For this review, use the dimensioned drawing (mm, ordinates from the lowest corner) and the shaded views. A direction names the side the tool comes from. Coordinates: 2 decimals unless noted, no trailing zeros. Write each loop counter-clockwise with the first axis right and the second up, starting at its lowest first coordinate (ties: lowest second). Pieces come first, ordered by that corner, then holes. Notation, with made-up numbers: M -12.75,36.5 L -5.75,36.5 A19 ccw -5.75,69.5 Z; hole C -15.75,-33.75 d5. An arc over 180 degrees is marked long. One line per question, with ' | ' between items.
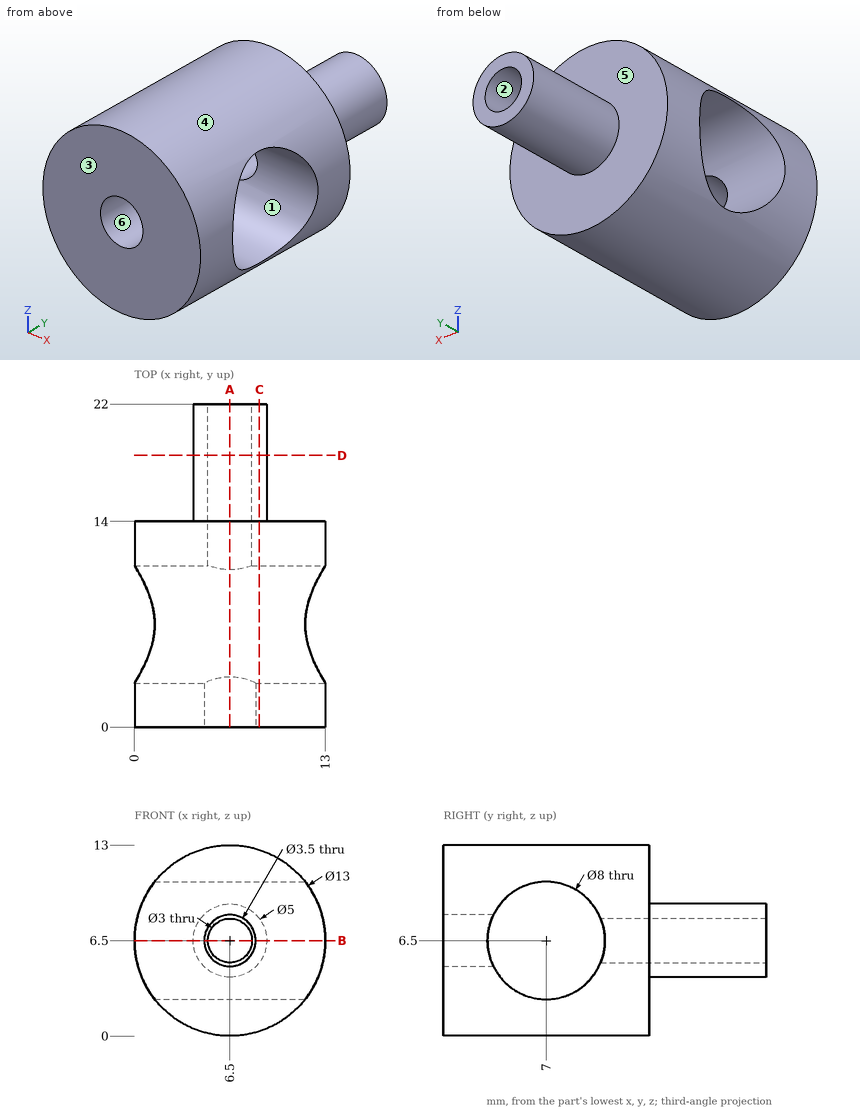
1. Draft analysis for pull direction Y (two halves, no side actions). For the marked faces 1, 2 and 3, state which applies: pulls with the +Y half, pulls with the -Y half, needs draft (parallel to the pull), parting line crosses it, or undercut.
Answer sheet:
face 1: undercut | face 2: needs draft | face 3: pulls with the -Y half
2. Insertion check: pin 1 Ø1 at (x, z) = (11.5, 3) entering from +Y; pin 2 Ø5 at (y, z) = (7, 6.5) entering from -X; pin 3 Ø1.5 at (x, y) = (7.5, 11.5) entering from -Z. Each pin has a flat end and moves straight along its axis. Give the tip position at first contact, or say it passes through.
Answer sheet:
pin 1: y = 14 | pin 2: through | pin 3: z = 0
3. Take a section at C-C (x = 8.5). Write out the cut boundary in (y, z).
Answer sheet:
outline: M 0,0.32 L 14,0.32 L 14,5 L 22,5 L 22,8 L 14,8 L 14,12.68 L 0,12.68 Z; hole C 7,6.5 d8
4. To check wall thickness, follow line 1 along Y through (x, z) = (3.5, 6.5); line 2 along X through (y, z) = (1.15, 6.5); line 3 along Y through (x, z) = (2.5, 3.5). State the ranges of each line that lie inside material, in increasing order. Write a range as [from, to].
Answer sheet:
line 1: [0, 3], [11, 14] | line 2: [0, 4.75], [8.25, 13] | line 3: [0, 4.35], [9.65, 14]
5. Take a section at D-D (y = 18.5). Write out the cut boundary in (x, z), then the cut area to 3 significant figures.
Answer sheet:
outline: C 6.5,6.5 d5; hole C 6.5,6.5 d3 | area: 12.6 mm^2
6. Tool access review of the marked faces 4, 5 and 6: name each direction out of +Z, -Z, +X, -X, +Y, -Y from which nothing blocks a thin tool from reaching the whole face with its end or side.
Answer sheet:
face 4: +Y, -Y | face 5: +Y | face 6: -Y
7. Take a section at A-A (x = 6.5). Write out the cut boundary in (y, z).
Answer sheet:
outline: M 0,0 L 14,0 L 14,4 L 22,4 L 22,5 L 10.71,5 A4 cw 3.4,4.75 L 0,4.75 Z; M 0,8.25 L 3.4,8.25 A4 cw 10.71,8 L 22,8 L 22,9 L 14,9 L 14,13 L 0,13 Z
8. Take a section at B-B (z = 6.5). Write out the cut boundary in (x, y), then the cut area to 3 significant figures.
Answer sheet:
outline: M 0,0 L 4.75,0 L 4.75,3 L 0,3 Z; M 0,11 L 5,11 L 5,22 L 4,22 L 4,14 L 0,14 Z; M 8,11 L 13,11 L 13,14 L 9,14 L 9,22 L 8,22 Z; M 8.25,0 L 13,0 L 13,3 L 8.25,3 Z | area: 74.5 mm^2
